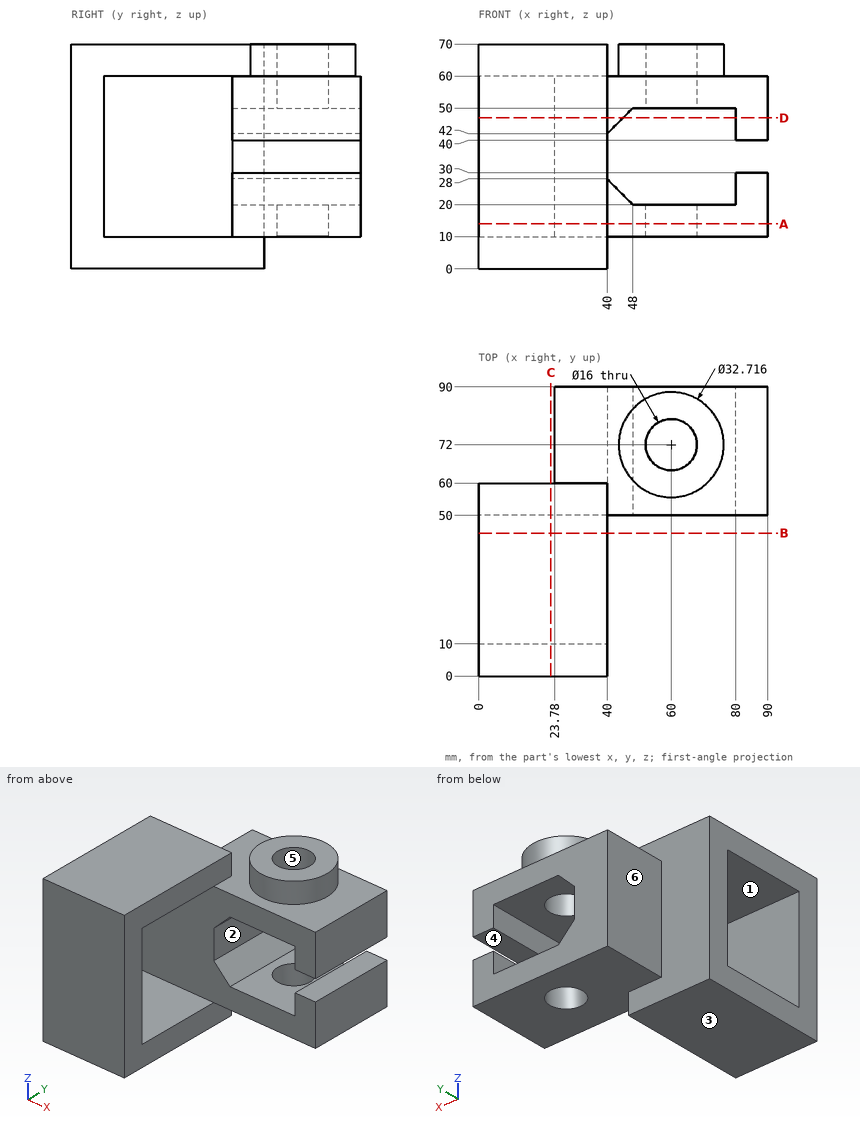
Can you work these out from the drawing? Everything is in mm from the part's minimum corner. A direction names the side the tool comes from. Round coordinates to 2 decimals unless told otherwise and drop trailing zeros. Order: outer loops, then holes, each group sorted by start corner. A loop starts at its lowest first (then second) coordinate and runs counter-clockwise, first axis right, second up. Notation, with made-up numbers: (6, 64) - (36, 64) arc R26 cw to (36, 85) - close; hole circle Ø6 at (-22, -5). An arc over 180 degrees is marked (long way). Answer in a Markdown table with one row per item.
(1) Suppose I cut it at A-A, the plane z = 14. Please give me the cut outline in (x, y).
From the geometry:
| item | result |
|---|---|
| outline | (0, 0) - (40, 0) - (40, 10) - (0, 10) - close; (0, 50) - (90, 50) - (90, 90) - (23.78, 90) - (23.78, 60) - (0, 60) - close; hole circle Ø16 at (60, 72) |
(2) Suppose I cut it at D-D, the plane z = 47. Please give me the cut outline in (x, y).
From the geometry:
| item | result |
|---|---|
| outline | (0, 0) - (40, 0) - (40, 10) - (0, 10) - close; (0, 50) - (45, 50) - (45, 90) - (23.78, 90) - (23.78, 60) - (0, 60) - close; (80, 50) - (90, 50) - (90, 90) - (80, 90) - close |
(3) If we mould it in two halves opening along X, with no side actions, what happens to the marked faces 4, 5 and 6? For each: released by +X, released by -X, zero draft, split by the parting line, or undercut.
From the geometry:
| item | result |
|---|---|
| face 4 | zero draft |
| face 5 | undercut |
| face 6 | released by -X |
(4) For P1, Ø11, axis at y = 79.5, z = 46, coming from the -X side; P2, Ø11, axis at x = 82.5, y = 72, coming from the -Z side; P3, Ø5, axis at x = 84, y = 66, coming from the +Z side, each with a flat end and sliding along its axis, tell me the tip position at first contact or that it passes through.
From the geometry:
| item | result |
|---|---|
| P1 | stops at x = 23.78 |
| P2 | stops at z = 10 |
| P3 | stops at z = 60 |
(5) Which directions (+Z, -Z, +X, -X, +Y, -Y) give clear straight access to the entire face, cutting with the end or side of a thin tool? Please do the marked faces 1, 2 and 3.
From the geometry:
| item | result |
|---|---|
| face 1 | +X, -X |
| face 2 | +Y, -Y |
| face 3 | -Z, +X, -X, +Y, -Y |
(6) Suppose I cut it at B-B, the plane y = 44.5. Please give me the cut outline in (x, z).
From the geometry:
| item | result |
|---|---|
| outline | (0, 0) - (40, 0) - (40, 10) - (0, 10) - close; (0, 60) - (40, 60) - (40, 70) - (0, 70) - close |
(7) Please list where these lines run through material, in increasing order: L1, parallel to Y at x = 60, z = 62.25; L2, parallel to Z at x = 29.5, y = 31; L3, parallel to Y at x = 60, z = 16. Write a range as from..to.
From the geometry:
| item | result |
|---|---|
| L1 | y = 55.64..64, 80..88.36 |
| L2 | z = 0..10, 60..70 |
| L3 | y = 50..64, 80..90 |
(8) Suppose I cut it at C-C, the plane x = 22.5. Please give me the cut outline in (y, z).
From the geometry:
| item | result |
|---|---|
| outline | (0, 0) - (60, 0) - (60, 70) - (0, 70) - close; hole (10, 10) - (50, 10) - (50, 60) - (10, 60) - close |
